Can you work these out from the drawing? Everything is in mm from the part's minimum corner. A direction names the side the tool comes from. Round coordinates to 2 decimals unless told otherwise and drop trailing zeros. Loops run counter-clockwise (first coordinate to the right, second up) from the corner with the lowest first, then second, coordinate; pieces in that order, holes last. Notation, with made-up numbers: (38, 33) -> (47, 33) arc R30 ccw to (47, 62) -> close; hole circle Ø6 at (6, -33.75). An arc over 180 degrees is marked (long way). Answer as a JSON object with one key per item and string values.
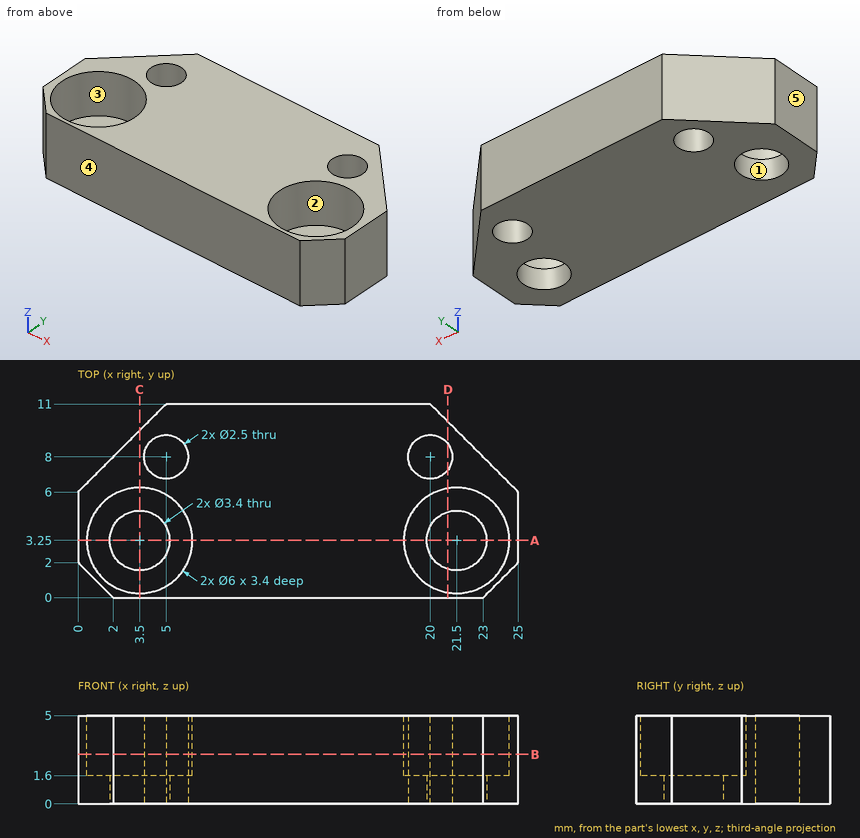
Q1. We'd pull the mould along Y, two halves only. Please class the marked faces 3, 4 and 5: pulls with the +Y half, pulls with the -Y half, needs draft (parallel to the pull), parting line crosses it, or undercut.
Determined:
{"face 3": "undercut", "face 4": "pulls with the -Y half", "face 5": "needs draft"}
Q2. On a 3-axis mill with a long thin cutter (end or side, diameter ignored), from which of +Z, -Z, +X, -X, +Y, -Y can I reach the whole of each face in a straight line? I mean the marked faces 1 and 2. Say none if no direction works.
Determined:
{"face 1": "+Z, -Z", "face 2": "+Z"}
Q3. I want a section at D-D, the plane x = 21. Write out the boundary of the cut face in (y, z), then the cut area to 3 significant figures.
Determined:
{"outline": "(0, 0) -> (1.63, 0) -> (1.63, 1.6) -> (0.29, 1.6) -> (0.29, 5) -> (0, 5) -> close; (4.87, 0) -> (7.25, 0) -> (7.25, 5) -> (6.21, 5) -> (6.21, 1.6) -> (4.87, 1.6) -> close; (8.75, 0) -> (10, 0) -> (10, 5) -> (8.75, 5) -> close", "area": "17.2 mm²"}
Q4. If I drill on L1, parallel to X at y = 0.75, z = 4.35; L2, parallel to X at y = 3.75, z = 0.3; L3, parallel to Y at x = 3.5, z = 0.85, over which ranges is the centre line in solid material (lowest first)? Write a range as [from, to].
Determined:
{"L1": "[1.25, 1.84], [5.16, 19.84], [23.16, 23.75]", "L2": "[0, 1.88], [5.12, 19.88], [23.12, 25]", "L3": "[0, 1.55], [4.95, 9.5]"}
Q5. I want a section at C-C, the plane x = 3.5. Write out the boundary of the cut face in (y, z), then the cut area to 3 significant figures.
Determined:
{"outline": "(0, 0) -> (1.55, 0) -> (1.55, 1.6) -> (0.25, 1.6) -> (0.25, 5) -> (0, 5) -> close; (4.95, 0) -> (9.5, 0) -> (9.5, 5) -> (6.25, 5) -> (6.25, 1.6) -> (4.95, 1.6) -> close", "area": "21.7 mm²"}
Q6. I want a section at B-B, the plane z = 2.8. Write out the boundary of the cut face in (x, y), then the cut area to 3 significant figures.
Determined:
{"outline": "(0, 2) -> (2, 0) -> (23, 0) -> (25, 2) -> (25, 6) -> (20, 11) -> (5, 11) -> (0, 6) -> close; hole circle Ø6 at (3.5, 3.25); hole circle Ø2.5 at (5, 8); hole circle Ø6 at (21.5, 3.25); hole circle Ø2.5 at (20, 8)", "area": "180 mm²"}
Q7. I'm going to push flat-ended pins straight in: pin 1 (5 mm diameter, centred on x = 3.5, y = 3.25, fed in from +Z); pin 2 (3 mm diameter, centred on x = 5, y = 8, fed in from +Z). Where does each tip first touch, or does it pass through?
Determined:
{"pin 1": "z = 1.6", "pin 2": "z = 5"}
Q8. I want a section at A-A, the plane y = 3.25. Write out the boundary of the cut face in (x, z).
Determined:
{"outline": "(0, 0) -> (1.8, 0) -> (1.8, 1.6) -> (0.5, 1.6) -> (0.5, 5) -> (0, 5) -> close; (5.2, 0) -> (19.8, 0) -> (19.8, 1.6) -> (18.5, 1.6) -> (18.5, 5) -> (6.5, 5) -> (6.5, 1.6) -> (5.2, 1.6) -> close; (23.2, 0) -> (25, 0) -> (25, 5) -> (24.5, 5) -> (24.5, 1.6) -> (23.2, 1.6) -> close"}
